Source: CAD feature listing. Evaluate the final solid. Frame: model axes, mm. Coordinates: 2 decimals unless noted, no trailing zeros. Order: outer loops, then holes, each group sorted by start corner. A loop starts at its lowest first (then second) coordinate and runs counter-clockwise, first axis right, second up.
Item 1: Section A-A on x = 45. Return the cut outline in (y, z).
Item 2: Ray query, line 1 (X direction, y = 7, z = -65); line 2 (Z direction, x = -45, y = 7.25); line 3 (Z direction, x = 37, y = 0.75). Return the intervals inside material, ascending.
Item 3: Section C-C on z = 58. Return the cut outline in (x, y), then the cut area to 3 significant figures.
Item 4: Section B-B on z = -65. Return the cut outline in (x, y).
Item 5: Contact query for flat-ended pins moving along their axis: P1, Ø7, axis at x = 45, z = 65, coming from the -Y side; P2, Ø0.8, axis at y = 0.5, z = -61, coming from the +X side; P3, Ø0.8, axis at x = -43, y = 0.5, coming from the -Z side. Output: stop coordinate, or through.
from build123d import *

# Parameters (mm, degrees)
SKETCH1_W                  = 110
SKETCH1_H                  = 150
BOSS_EXTRUDE1_DEPTH        = 10
SKETCH2_W                  = 20
SKETCH2_H                  = 20
CUT_EXTRUDE1_DEPTH         = 1
F_4_5_4_5_DIAMETER_HOLE1_D = 4.5
FILLET1_R                  = 1
FILLET2_R                  = 1


with BuildPart() as part:
    # Sketch1 → Boss-Extrude1 (new body)
    with BuildSketch(Plane(origin=(0, 0, 0), x_dir=(1, 0, 0), z_dir=(0, 1, 0))):
        Rectangle(SKETCH1_W, SKETCH1_H)
    extrude(amount=BOSS_EXTRUDE1_DEPTH)

    # Sketch2 → Cut-Extrude1 (cut)
    with BuildSketch(Plane.XZ):
        with Locations((-45, 65)):
            Rectangle(SKETCH2_W, SKETCH2_H)
        with Locations((45, 65)):
            Rectangle(SKETCH2_W, SKETCH2_H)
        with Locations((45, -65)):
            Rectangle(SKETCH2_W, SKETCH2_H)
        with Locations((-45, -65)):
            Rectangle(SKETCH2_W, SKETCH2_H)
    extrude(amount=-CUT_EXTRUDE1_DEPTH, mode=Mode.SUBTRACT)

    # Ø4.5 (4.5) Diameter Hole1 (through all)
    with Locations(Plane(origin=(0, 1, 0), x_dir=(-1, 0, 0), z_dir=(0, -1, 0))):
        with Locations((-45, 65), (45, 65), (45, -65), (-45, -65)):
            Hole(F_4_5_4_5_DIAMETER_HOLE1_D / 2)

    # Fillet1
    fillet1_edges = [part.edges().sort_by_distance(p)[0] for p in [
        (-35, 0.5, -55),
        (35, 0.5, -55),
        (35, 0.5, 55),
        (-35, 0.5, 55),
    ]]
    fillet(fillet1_edges, radius=FILLET1_R)

    # Fillet2
    fillet2_edges = [part.edges().sort_by_distance(p)[0] for p in [
        (-55, 5.5, -75),
        (-55, 5.5, 75),
        (55, 5.5, 75),
        (55, 5.5, -75),
    ]]
    fillet(fillet2_edges, radius=FILLET2_R)


solid = part.part
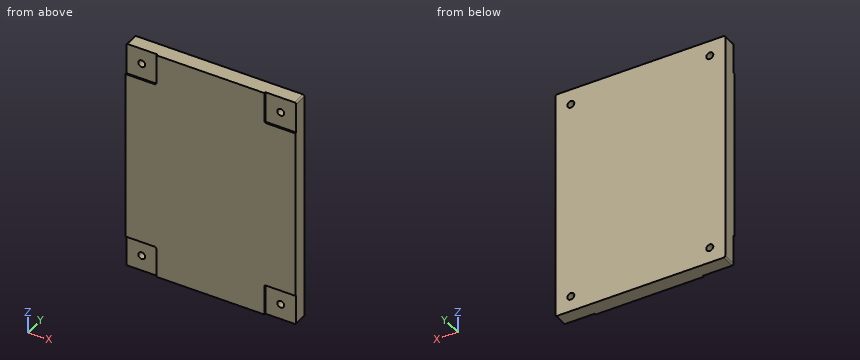
Answer list:
1. outline: (0, -55) - (1, -55) - (1, -62.75) - (10, -62.75) - (10, 62.75) - (1, 62.75) - (1, 55) - (0, 55) - close; (1, -75) - (10, -75) - (10, -67.25) - (1, -67.25) - close; (1, 67.25) - (10, 67.25) - (10, 75) - (1, 75) - close
2. line 1: x = -55 to -47.25, -42.75 to 42.75, 47.25 to 55
2. line 2: z = -75 to -67.25, -62.75 to 62.75, 67.25 to 75
2. line 3: z = -55 to 55
3. outline: (-55, 1) - (-35, 1) - (-35, 0) - (35, 0) - (35, 1) - (55, 1) - (55, 10) - (-55, 10) - close
3. area: 1,060 mm2
4. outline: (-55, 1) - (-47.25, 1) - (-47.25, 10) - (-55, 10) - close; (-42.75, 1) - (-35, 1) - (-35, 0) - (35, 0) - (35, 1) - (42.75, 1) - (42.75, 10) - (-42.75, 10) - close; (47.25, 1) - (55, 1) - (55, 10) - (47.25, 10) - close
5. P1: stops at y = 1
5. P2: stops at x = 35
5. P3: stops at z = -55
